```python
from build123d import *

# Parameters (mm, degrees)
SKETCH_1_R                = 35
EXTRUDE_1_DEPTH           = 8
HOLE_WIZARD_1_D           = 5.5
HOLE_WIZARD_1_CBORE_D     = 10
HOLE_WIZARD_1_CBORE_DEPTH = 5.7
CHAMFER_1_SIZE            = 1


with BuildPart() as part:
    # 草图1 → 凸台-拉伸1 (new body)
    with BuildSketch(Plane.XY):
        Circle(SKETCH_1_R)
    extrude(amount=EXTRUDE_1_DEPTH)

    # 打孔尺寸根据内六角圆柱头螺钉的类型1 (through all)
    with Locations(Plane.XY.offset(8)):
        with Locations((0, 17.5), (0, -17.5)):
            CounterBoreHole(HOLE_WIZARD_1_D / 2, HOLE_WIZARD_1_CBORE_D / 2, HOLE_WIZARD_1_CBORE_DEPTH)

    # 倒角1
    chamfer_1_edges = [part.edges().sort_by_distance(p)[0] for p in [
        (-35, 0, 0),
        (-35, 0, 8),
    ]]
    chamfer(chamfer_1_edges, length=CHAMFER_1_SIZE)


solid = part.part
```
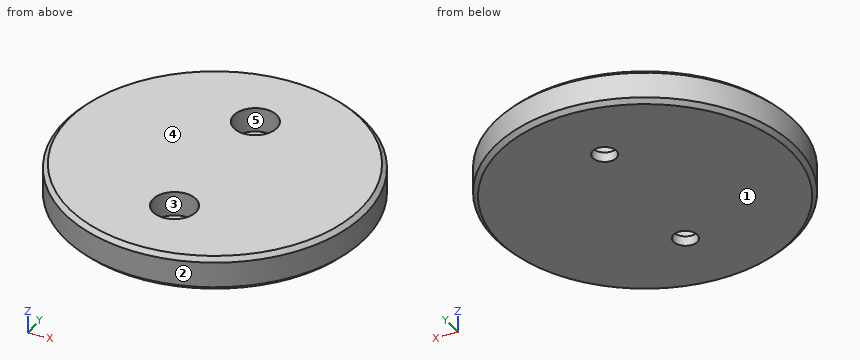
Geometry: final body of the model. Coordinates: model frame, mm. Face numbers are marked on the shaded views. A direction names the side the tool comes from. Give positions to 0.01 mm unless a question says otherwise; leave off trailing zeros. Loops run counter-clockwise (first coordinate to the right, second up) from the corner with the lowest first, then second, coordinate; pieces in that order, holes last. Notation, with made-up numbers: (-13, 28) - (35, 28) arc R35 cw to (35, 61) - close; hole circle Ø5 at (68, -24). An arc over 180 degrees is marked (long way). Answer as CSV lines item,"result". Start each with the question number.
(1) Section query A-A (x = 0). Output: boundary loops of the cut face in (y, z), and give its area (3 significant figures).
(2) Section query B-B (z = 3.75). Output: boundary loops of the cut face in (x, y), and give its area (3 significant figures).
(3) Mould query, pull axis X, two halves, no side actions, for the marked faces 1, 2 and 3. Classes: +X half, -X half, draft (parallel to the pull), parting line (faces both ways), or undercut.
(4) Ray query, line 1 along Y through (x, z) = (0, 1.8); line 2 along Y through (x, z) = (0, 0.5); line 3 along X through (y, z) = (2.5, 3). Return the intervals inside material, ascending. Write a range as [from, to].
(5) Pin query (flat end, axial travel): P1, Ø3, axis at x = 22, z = 4, coming from the -Y side; P2, Ø11, axis at x = -1.5, y = -19.5, coming from the +Z side; P3, Ø8, axis at x = 0, y = -17.5, coming from the +Z side; P4, Ø4, axis at x = 17, z = 6.5, coming from the -Y side. Return the tip coordinate at first contact, or that it passes through.
(6) Reachability of the marked faces 4 and 5 from +Z, -Z, +X, -X, +Y, -Y: full face, straight path, thin tool, end or side. Return the list, or none.
Worked answers:
1,outline,"(-35, 1) - (-34, 0) - (-20.25, 0) - (-20.25, 2.3) - (-22.5, 2.3) - (-22.5, 8) - (-34, 8) - (-35, 7) - close; (-14.75, 0) - (14.75, 0) - (14.75, 2.3) - (12.5, 2.3) - (12.5, 8) - (-12.5, 8) - (-12.5, 2.3) - (-14.75, 2.3) - close; (20.25, 0) - (34, 0) - (35, 1) - (35, 7) - (34, 8) - (22.5, 8) - (22.5, 2.3) - (20.25, 2.3) - close"
1,area,"419 mm^2"
2,outline,"circle Ø70 at (0, 0); hole circle Ø10 at (0, -17.5); hole circle Ø10 at (0, 17.5)"
2,area,"3,690 mm^2"
3,face 1,"draft"
3,face 2,"parting line"
3,face 3,"undercut"
4,line 1,"y = [-35, -20.25], [-14.75, 14.75], [20.25, 35]"
4,line 2,"y = [-34.5, -20.25], [-14.75, 14.75], [20.25, 34.5]"
4,line 3,"x = [-34.91, 34.91]"
5,P1,"stops at y = -28.37"
5,P2,"stops at z = 8"
5,P3,"stops at z = 2.3"
5,P4,"stops at y = -31.62"
6,face 4,"+Z, +X, -X, +Y, -Y"
6,face 5,"+Z"
